Input: part model. Units: mm. Frame: model coordinates. Face numbers are marked on the shaded views. A direction names the side the tool comes from. Coordinates: 2 decimals unless noted, no trailing zeros. Loops run counter-clockwise (first coordinate to the right, second up) from the corner with the lowest first, then second, coordinate; pieces in that order, holes last.
Item 1: Reachability of the marked faces 5, 6, 7 and 8 from +Z, -Z, +X, -X, +Y, -Y: full face, straight path, thin tool, end or side. Return the list, or none.
Item 2: Pull-direction query (X, two-part tool) for the marked faces 1, 2, 3 and 4; classes: released by +X, released by -X, zero draft, split by the parting line, or undercut.
Item 3: Section A-A on y = 9. Return loops of the section in (x, z).
Item 4: Section C-C on x = 2. Return loops of the section in (y, z).
Item 5: Section D-D on z = 3.5. Return loops of the section in (x, y), and give its area (3 significant figures).
Item 6: Contact query for flat-ended pins moving along their axis: P1, Ø6, axis at y = 19, z = 33, coming from the +X side; P2, Ø6.5, axis at y = 15, z = 1.5, coming from the -X side; P3, Ø6, axis at x = -20.5, z = 26.5, coming from the +Y side. Output: stop coordinate, or through.
Item 7: Ray query, line 1 along Z through (x, y) = (-18.5, 23.5); line 2 along Y through (x, z) = (-44.5, 19); line 3 along Z through (x, y) = (17, 5). Return the intervals inside material, ascending.
Item 8: Section B-B on y = 30.5. Return loops of the section in (x, z), and give its area (3 significant figures).
```python
from build123d import *

# Parameters (mm, degrees)
CLEVIS_EAR_1_DEPTH         = 6
BASE_PLATE_DEPTH           = 6
MOUNTING_HOLES_SKETCH_R    = 6.5
MOUNTING_HOLES_2X_13_DEPTH = 67.717997207
CLEVIS_EAR_2_DEPTH         = 6


with BuildPart() as part:
    # Clevis Ear 1 Sketch → Clevis Ear 1 (new body)
    with BuildSketch(Plane.XY):
        with BuildLine():
            Line((-27.211796247, 0), (7.788203753, 0))
            Line((7.788203753, 0), (7.788203753, 32))
            ThreePointArc((7.788203753, 32), (6.909524097, 34.121320344), (4.788203753, 35))
            Line((4.788203753, 35), (-3.211796247, 35))
            Line((-3.211796247, 35), (-3.211796247, 23))
            ThreePointArc((-3.211796247, 23), (-9.711796247, 16.5), (-16.211796247, 23))
            Line((-16.211796247, 23), (-16.211796247, 35))
            Line((-16.211796247, 35), (-24.211796247, 35))
            ThreePointArc((-24.211796247, 35), (-26.33311659, 34.121320344), (-27.211796247, 32))
            Line((-27.211796247, 32), (-27.211796247, 0))
        make_face()
    extrude(amount=CLEVIS_EAR_1_DEPTH)

    # Base Plate Sketch → Base Plate (add)
    with BuildSketch(Plane.XZ):
        with BuildLine():
            Line((-35.558376082, 5.974380222), (14.441623918, 5.974380222))
            ThreePointArc((14.441623918, 5.974380222), (28.441623918, 19.974380222), (14.441623918, 33.974380222))
            Line((14.441623918, 33.974380222), (-35.558376082, 33.974380222))
            ThreePointArc((-35.558376082, 33.974380222), (-49.558376082, 19.974380222), (-35.558376082, 5.974380222))
        make_face()
    extrude(amount=-BASE_PLATE_DEPTH)

    # Mounting Holes Sketch → Mounting Holes 2xØ13 (cut, through all)
    with BuildSketch(Plane(origin=(0, 6, 0), x_dir=(1, 0, 0), z_dir=(0, 1, 0))):
        with Locations(Location((-35.558376082, -19.974380222, 0), (0, 0, 270))):
            Circle(MOUNTING_HOLES_SKETCH_R)
        with Locations(Location((14.441623918, -19.974380222, 0), (0, 0, 270))):
            Circle(MOUNTING_HOLES_SKETCH_R)
    extrude(amount=-MOUNTING_HOLES_2X_13_DEPTH, mode=Mode.SUBTRACT)

    # Clevis Ear 2 Sketch → Clevis Ear 2 (add)
    with BuildSketch(Plane.XY.offset(33.974380222)):
        with BuildLine():
            Line((-27.211796247, 0), (7.788203753, 0))
            Line((7.788203753, 0), (7.788203753, 32))
            ThreePointArc((7.788203753, 32), (6.909524097, 34.121320344), (4.788203753, 35))
            Line((4.788203753, 35), (-3.211796247, 35))
            Line((-3.211796247, 35), (-3.211796247, 23))
            ThreePointArc((-3.211796247, 23), (-9.711796247, 16.5), (-16.211796247, 23))
            Line((-16.211796247, 23), (-16.211796247, 35))
            Line((-16.211796247, 35), (-24.211796247, 35))
            ThreePointArc((-24.211796247, 35), (-26.33311659, 34.121320344), (-27.211796247, 32))
            Line((-27.211796247, 32), (-27.211796247, 0))
        make_face()
    extrude(amount=CLEVIS_EAR_2_DEPTH)


solid = part.part
```
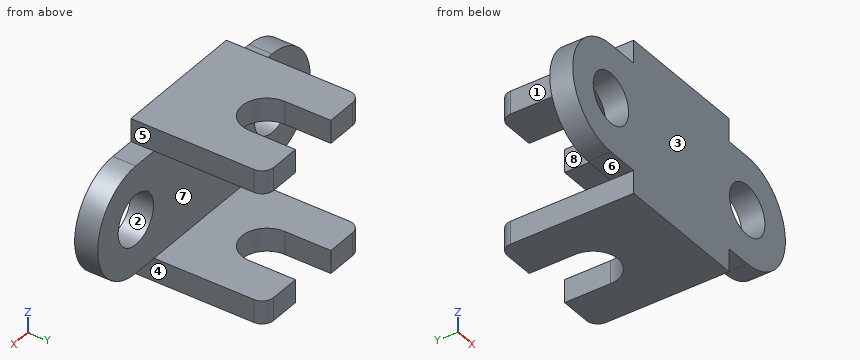
Results found:
1. face 5: +Z, +X, +Y, -Y
1. face 6: -Z, -X, +Y, -Y
1. face 7: +X, -X, +Y
1. face 8: +Z, -Z, +Y
2. face 1: released by -X
2. face 2: undercut
2. face 3: zero draft
2. face 4: released by +X
3. outline: (-27.21, 0) - (7.79, 0) - (7.79, 6) - (-27.21, 6) - close; (-27.21, 33.97) - (7.79, 33.97) - (7.79, 39.97) - (-27.21, 39.97) - close
4. outline: (0, 0) - (35, 0) - (35, 6) - (6, 6) - (6, 33.97) - (35, 33.97) - (35, 39.97) - (0, 39.97) - close
5. outline: (-27.21, 0) - (7.79, 0) - (7.79, 32) arc R3 ccw to (4.79, 35) - (-3.21, 35) - (-3.21, 23) arc R6.5 cw to (-16.21, 23) - (-16.21, 35) - (-24.21, 35) arc R3 ccw to (-27.21, 32) - close
5. area: 999 mm2
6. P1: stops at x = 7.79
6. P2: stops at x = -27.21
6. P3: stops at y = 6
7. line 1: z = 0 to 6, 33.97 to 39.97
7. line 2: y = 0 to 6
7. line 3: z = 6.21 to 14, 25.95 to 33.74
8. outline: (-27.21, 0) - (-16.21, 0) - (-16.21, 6) - (-27.21, 6) - close; (-27.21, 33.97) - (-16.21, 33.97) - (-16.21, 39.97) - (-27.21, 39.97) - close; (-3.21, 0) - (7.79, 0) - (7.79, 6) - (-3.21, 6) - close; (-3.21, 33.97) - (7.79, 33.97) - (7.79, 39.97) - (-3.21, 39.97) - close
8. area: 264 mm2
